For this review, take the finished solid that the model builds, in its own axes (mm). A direction names the side the tool comes from. Give positions to 0.01 mm unless a question says otherwise; leave off trailing zeros. Order: outer loops, then holes, each group sorted by start corner. A loop starts at its lowest first (then second) coordinate and runs counter-clockwise, first axis right, second up. Notation, with made-up numbers: (16, 45.25) - (58, 45.25) arc R31 cw to (58, 79.25) - close; hole circle Ø5 at (-24, 12). An arc over 180 degrees is marked (long way). One line per item, written item: value.
```python
from build123d import *

# Parameters (mm, degrees)
BASE_PLATE_SKETCH_W     = 38
BASE_PLATE_SKETCH_H     = 92
BASE_PLATE_DEPTH        = 13
MAIN_BODY_104MM_DEPTH   = 104
CURVED_RELIEF_CUT_DEPTH = 13
SLOT_CUT_DEPTH          = 13
GUSSET_BOSS_38MM_DEPTH  = 38
NOTCH_CUT_A_DEPTH       = 16
NOTCH_CUT_B_DEPTH       = 16


with BuildPart() as part:
    # Base Plate Sketch → Base Plate (new body)
    with BuildSketch(Plane.XY):
        with Locations((19, -46)):
            Rectangle(BASE_PLATE_SKETCH_W, BASE_PLATE_SKETCH_H)
    extrude(amount=BASE_PLATE_DEPTH)

    # Main Body Profile Sketch → Main Body 104mm (add)
    with BuildSketch(Plane.ZY):
        Polygon((13, -4), (100.5, -4), (100.5, -8), (113.5, -8), (113.5, -4), (129, -4), (129, -17), (13, -17), align=None)
    extrude(amount=-MAIN_BODY_104MM_DEPTH)

    # Curved Relief Sketch → Curved Relief Cut (cut)
    with BuildSketch(Plane.XZ.offset(17)):
        with BuildLine():
            Line((104, 88), (104, 13))
            Line((104, 13), (29, 13))
            ThreePointArc((29, 13), (50.966991411, 66.033008589), (104, 88))
        make_face()
    extrude(amount=-CURVED_RELIEF_CUT_DEPTH, mode=Mode.SUBTRACT)

    # Slot Sketch → Slot Cut (cut)
    with BuildSketch(Plane.XZ.offset(17)):
        with BuildLine():
            Line((26, 113.5), (76, 113.5))
            ThreePointArc((76, 113.5), (82.5, 107), (76, 100.5))
            Line((76, 100.5), (26, 100.5))
            ThreePointArc((26, 100.5), (19.5, 107), (26, 113.5))
        make_face()
    extrude(amount=-SLOT_CUT_DEPTH, mode=Mode.SUBTRACT)

    # Gusset Boss Sketch → Gusset Boss 38mm (add)
    with BuildSketch(Plane.ZY):
        Polygon((13, -17), (76, -17), (13, -86), align=None)
    extrude(amount=-GUSSET_BOSS_38MM_DEPTH)

    # Notch Cut A Sketch → Notch Cut A (cut)
    with BuildSketch(Plane(origin=(38, 0, 0), x_dir=(0, 0, -1), z_dir=(1, 0, 0))):
        Polygon((-76, -17), (-13, -17), (-13, -86), align=None)
    extrude(amount=-NOTCH_CUT_A_DEPTH, mode=Mode.SUBTRACT)

    # Notch Cut B Sketch → Notch Cut B (cut)
    with BuildSketch(Plane.ZY):
        Polygon((76, -17), (13, -86), (13, -17), align=None)
    extrude(amount=-NOTCH_CUT_B_DEPTH, mode=Mode.SUBTRACT)


solid = part.part
```
(1) Take a section at D-D (x = 49). Write out the cut boundary in (y, z), then the cut area to 3 significant figures.
Answers below:
outline: (-17, 63.99) - (-4, 63.99) - (-4, 100.5) - (-17, 100.5) - close; (-17, 113.5) - (-4, 113.5) - (-4, 129) - (-17, 129) - close
area: 676 mm^2
(2) Take a section at A-A (z = 110.5). Write out the cut boundary in (x, y), then the cut area to 3 significant figures.
Answers below:
outline: (0, -17) - (20.52, -17) - (20.52, -8) - (0, -8) - close; (81.48, -17) - (104, -17) - (104, -8) - (81.48, -8) - close
area: 387 mm^2
(3) For P1, Ø1.5, axis at x = 31.5, y = -68, coming from the -Z side; P2, Ø10, axis at y = -16, z = 42.5, coming from the +X side; P3, Ø6.5, axis at x = 85, z = 107, coming from the +Y side; P4, Ø2, axis at x = 29.5, z = 32, coming from the +Y side, all flat-tipped, find the tip position at first contact; note any pin that passes through.
Answers below:
P1: stops at z = 0
P2: stops at x = 37.41
P3: stops at y = -8
P4: stops at y = -4
(4) Wall thickness on line 1 (Z direction, x = 4, y = -23); line 2 (X direction, y = -62, z = 7.5); line 3 (Y direction, x = 27, z = 16.5): over which ranges is each line inside the solid? List them lowest first. Write a range as from..to.
Answers below:
line 1: z = 0..13
line 2: x = 0..38
line 3: y = -17..-4
(5) Take a section at B-B (x = 13.5). Write out the cut boundary in (y, z).
Answers below:
outline: (-92, 0) - (0, 0) - (0, 13) - (-4, 13) - (-4, 100.5) - (-8, 100.5) - (-8, 113.5) - (-4, 113.5) - (-4, 129) - (-17, 129) - (-17, 13) - (-92, 13) - close
(6) Machinability: for faces 1 (the face through (82.5, -12.6, 107.1)), 2 (the face through (51, -4, 121)), 3 (the face through (51, -9, 100.5)), 4 (the face through (10, -8, 107)), 5 (the face through (38, -45, 7)), which of the approach directions +Z, -Z, +X, -X, +Y, -Y give a long, thin tool a straight path to every point of the face, cutting with its end or side? Answer none if there is none.
Answers below:
face 1: +Y, -Y
face 2: +Z, +X, -X, +Y
face 3: +Y
face 4: +X, -X, +Y
face 5: -Z, +X, +Y, -Y
(7) Take a section at C-C (y = -79). Write out the cut boundary in (x, z), then the cut area to 3 significant figures.
Answers below:
outline: (0, 0) - (38, 0) - (38, 13) - (22, 13) - (22, 19.39) - (16, 19.39) - (16, 13) - (0, 13) - close
area: 532 mm^2
